Geometry: see drawing. Coordinates: mm, zero at the bounding-box minimum. Round coordinates to 2 decimals unless told otherwise and drop trailing zeros. Loops run counter-clockwise (first coordinate to the right, second up) from the corner with the lowest first, then second, coordinate; pieces in that order, holes last. Notation, with made-up numbers: (87, 72.25) -> (119, 72.25) arc R14 ccw to (119, 95.25) -> close; hole circle Ø7 at (23.5, 63.25). An arc over 180 degrees is marked (long way). Answer in a Markdown table with one row per item.
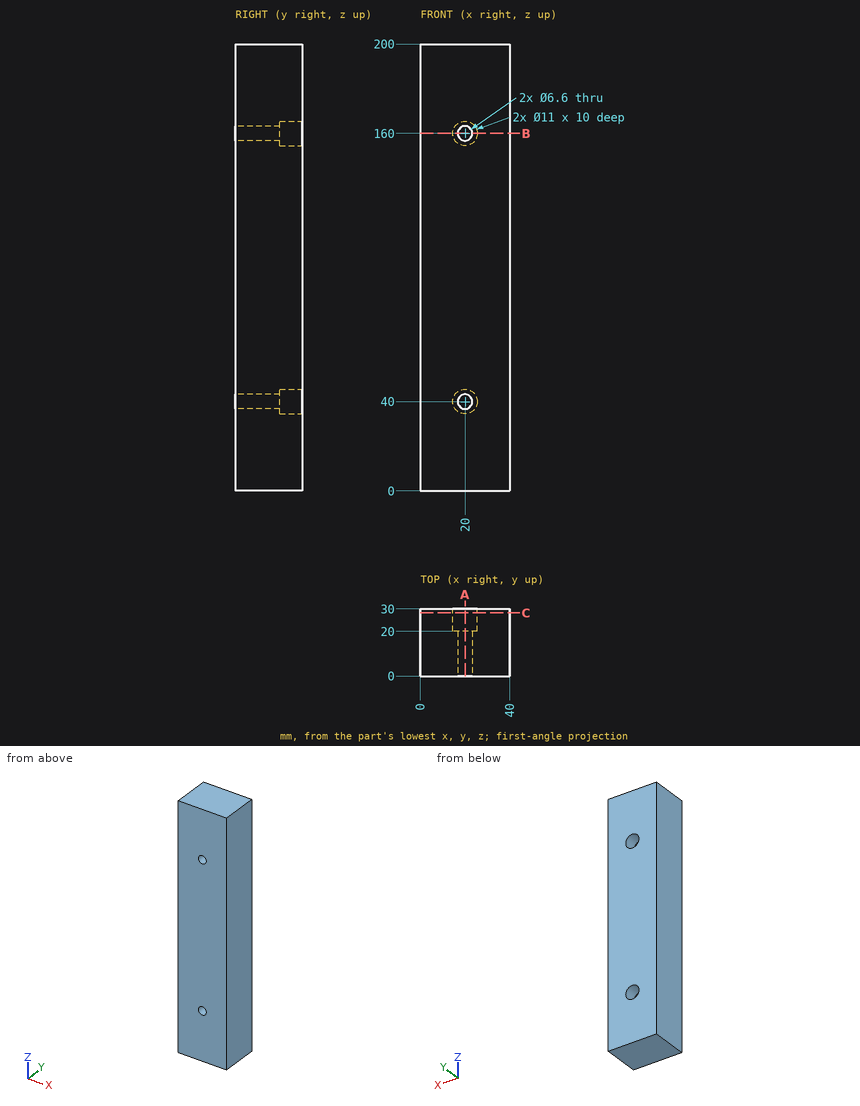
Item 1: Section query C-C, the plane y = 28.25. Output: boundary loops of the cut face in (x, z), and give its area (3 significant figures).
Ans:
| item | result |
|---|---|
| outline | (0, 0) -> (40, 0) -> (40, 200) -> (0, 200) -> close; hole circle Ø11 at (20, 40); hole circle Ø11 at (20, 160) |
| area | 7,810 mm2 |
Item 2: Section query B-B, the plane z = 160. Output: boundary loops of the cut face in (x, y), and give its area (3 significant figures).
Ans:
| item | result |
|---|---|
| outline | (0, 0) -> (16.7, 0) -> (16.7, 20) -> (14.5, 20) -> (14.5, 30) -> (0, 30) -> close; (23.3, 0) -> (40, 0) -> (40, 30) -> (25.5, 30) -> (25.5, 20) -> (23.3, 20) -> close |
| area | 958 mm2 |
Item 3: Section query A-A, the plane x = 20. Output: boundary loops of the cut face in (y, z).
Ans:
| item | result |
|---|---|
| outline | (0, 0) -> (30, 0) -> (30, 34.5) -> (20, 34.5) -> (20, 36.7) -> (0, 36.7) -> close; (0, 43.3) -> (20, 43.3) -> (20, 45.5) -> (30, 45.5) -> (30, 154.5) -> (20, 154.5) -> (20, 156.7) -> (0, 156.7) -> close; (0, 163.3) -> (20, 163.3) -> (20, 165.5) -> (30, 165.5) -> (30, 200) -> (0, 200) -> close |
Item 4: Ray query, L1, parallel to Z at x = 20, y = 22.75; L2, parallel to X at y = 27.5, z = 40; L3, parallel to X at y = 13.75, z = 160. Return the intervals inside material, ascending.
Ans:
| item | result |
|---|---|
| L1 | 0 to 34.5, 45.5 to 154.5, 165.5 to 200 |
| L2 | 0 to 14.5, 25.5 to 40 |
| L3 | 0 to 16.7, 23.3 to 40 |
